```python
from build123d import *

# Parameters (mm, degrees)
SKETCH2_R           = 2.93
BOSS_EXTRUDE1_DEPTH = 3
SKETCH3_R           = 1.5
BOSS_EXTRUDE2_DEPTH = 12
CUT_EXTRUDE1_DEPTH  = 1.3


with BuildPart() as part:
    # Sketch2 → Boss-Extrude1 (new body)
    with BuildSketch(Plane(origin=(0, 0, 0), x_dir=(1, 0, 0), z_dir=(0, 1, 0))):
        with Locations(Location((0, 0, 0), (0, 0, 270))):
            Circle(SKETCH2_R)
    extrude(amount=BOSS_EXTRUDE1_DEPTH)

    # Sketch3 → Boss-Extrude2 (add)
    with BuildSketch(Plane(origin=(0, 3, 0), x_dir=(1, 0, 0), z_dir=(0, 1, 0))):
        with Locations(Location((0, 0, 0), (0, 0, 270))):
            Circle(SKETCH3_R)
    extrude(amount=BOSS_EXTRUDE2_DEPTH)

    # Sketch4 → Cut-Extrude1 (cut)
    with BuildSketch(Plane.XZ):
        Polygon((0.989792051, 0.827291784), (-0.221559676, 1.270830953), (-1.211351727, 0.443539168), (-0.989792051, -0.827291784), (0.221559676, -1.270830953), (1.211351727, -0.443539168), align=None)
    extrude(amount=-CUT_EXTRUDE1_DEPTH, mode=Mode.SUBTRACT)


solid = part.part
```
Input: part model. Units: mm. Frame: model coordinates. A direction names the side the tool comes from. Round coordinates to 2 decimals unless told otherwise and drop trailing zeros. Order: outer loops, then holes, each group sorted by start corner. A loop starts at its lowest first (then second) coordinate and runs counter-clockwise, first axis right, second up. Notation, with made-up numbers: (81.25, 4.25) - (95.25, 4.25) arc R20 cw to (95.25, 40.25) - close; hole circle Ø5 at (3.5, 87). An arc over 180 degrees is marked (long way). Answer in a Markdown table with one row per item.
Item 1: Section query C-C (y = 6). Return the cut outline in (x, z).
Model answer:
| item | result |
|---|---|
| outline | circle Ø3 at (0, 0) |
Item 2: Pin query (flat end, axial travel): pin 1 (3 mm diameter, centred on y = 6, z = 0.5, fed in from +X); pin 2 (2 mm diameter, centred on x = 1.5, y = 13.5, fed in from -Z); pin 3 (2.5 mm diameter, centred on x = 0, z = 0, fed in from -Y); pin 4 (2 mm diameter, centred on y = 12, z = -1.5, fed in from -X). Return the tip coordinate at first contact, or that it passes through.
Model answer:
| item | result |
|---|---|
| pin 1 | stops at x = 1.5 |
| pin 2 | stops at z = -1.41 |
| pin 3 | stops at y = 0 |
| pin 4 | stops at x = -1.41 |
Item 3: Section query A-A (z = -0.15). Return the cut outline in (x, y), then the cut area to 3 significant figures.
Model answer:
| item | result |
|---|---|
| outline | (-2.93, 0) - (-1.11, 0) - (-1.11, 1.3) - (1.16, 1.3) - (1.16, 0) - (2.93, 0) - (2.93, 3) - (1.49, 3) - (1.49, 15) - (-1.49, 15) - (-1.49, 3) - (-2.93, 3) - close |
| area | 50.4 mm² |
Item 4: Line query: line 1 (Y direction, x = 1.85, z = 2.1); line 2 (Y direction, x = -0.55, z = -0.1); line 3 (X direction, y = 6.5, z = -0.8). Output: solid intervals per line, ascending.
Model answer:
| item | result |
|---|---|
| line 1 | y = 0 to 3 |
| line 2 | y = 1.3 to 15 |
| line 3 | x = -1.27 to 1.27 |
Item 5: Reachability of faces 4 (the flat face through (1.1, 0.6, 0.2)), 5 (the flat face through (0, 15, 0)), 6 (the flat face through (-1.3, 3, 1.3)) from +Z, -Z, +X, -X, +Y, -Y: full face, straight path, thin tool, end or side. Return the list, or none.
Model answer:
| item | result |
|---|---|
| face 4 | -Y |
| face 5 | +Z, -Z, +X, -X, +Y |
| face 6 | +Y |
Item 6: Section query D-D (y = 2.5). Return the cut outline in (x, z).
Model answer:
| item | result |
|---|---|
| outline | circle Ø5.86 at (0, 0) |
Item 7: Section query B-B (x = 0). Return the cut outline in (y, z), then the cut area to 3 significant figures.
Model answer:
| item | result |
|---|---|
| outline | (0, -2.93) - (3, -2.93) - (3, -1.5) - (15, -1.5) - (15, 1.5) - (3, 1.5) - (3, 2.93) - (0, 2.93) - (0, 1.19) - (1.3, 1.19) - (1.3, -1.19) - (0, -1.19) - close |
| area | 50.5 mm² |
Item 8: Mould query, pull axis Z, two halves, no side actions, for faces 1 (the flat face through (-1.3, 0, 0)), 2 (the flat face through (0.71, 0.64, -0.86)), 3 (the cylindrical face through (0.45, 8.92, 1.43)). Classes: released by +Z, released by -Z, zero draft, split by the parting line, or undercut.
Model answer:
| item | result |
|---|---|
| face 1 | zero draft |
| face 2 | undercut |
| face 3 | split by the parting line |
